from build123d import *

# Parameters (mm, degrees)
SKETCH1_W             = 12
SKETCH1_H             = 43.5
BOSS_EXTRUDE1_DEPTH   = 2
M3_TAPPED_HOLE1_D     = 2.5
M3_TAPPED_HOLE1_DEPTH = 7.5
M3_TAPPED_HOLE1_TIP   = 0.751075774
SKETCH6_W             = 25
SKETCH6_H             = 12
BOSS_EXTRUDE2_DEPTH   = 14
SKETCH7_W             = 25
SKETCH7_H             = 8
CUT_EXTRUDE4_DEPTH    = 32.273990791
SKETCH8_R             = 2.5
CUT_EXTRUDE5_DEPTH    = 15
SKETCH9_W             = 13
SKETCH9_H             = 4
SKETCH9_W_2           = 10
SKETCH9_H_2           = 6
CUT_EXTRUDE6_DEPTH    = 18
CHAMFER2_SIZE         = 2
FILLET1_R             = 2
FILLET2_R             = 2
SKETCH3_W             = 8
SKETCH3_H             = 8
CUT_EXTRUDE2_DEPTH    = 10
SKETCH10_R            = 0.25
CUT_EXTRUDE7_DEPTH    = 10
CUT_EXTRUDE8_DEPTH    = 10


with BuildPart() as part:
    # Sketch1 → Boss-Extrude1 (new body)
    with BuildSketch(Plane(origin=(0, 0, 0), x_dir=(1, 0, 0), z_dir=(0, 1, 0))):
        Rectangle(SKETCH1_W, SKETCH1_H)
    extrude(amount=BOSS_EXTRUDE1_DEPTH)

    # M3 Tapped Hole1
    with Locations(Plane(origin=(0, 2, 17.75), x_dir=(0, 0, 1), z_dir=(0, 1, 0))):
        with Locations((0, 0)):
            Hole(M3_TAPPED_HOLE1_D / 2, depth=M3_TAPPED_HOLE1_DEPTH)
            with Locations((0, 0, -(M3_TAPPED_HOLE1_DEPTH + M3_TAPPED_HOLE1_TIP / 2))):  # 118° drill point
                Cone(0, M3_TAPPED_HOLE1_D / 2, M3_TAPPED_HOLE1_TIP, mode=Mode.SUBTRACT)

    # Sketch6 → Boss-Extrude2 (add)
    with BuildSketch(Plane.XY.offset(21.75)):
        with Locations((-6.5, -4)):
            Rectangle(SKETCH6_W, SKETCH6_H)
    extrude(amount=-BOSS_EXTRUDE2_DEPTH)

    # Sketch7 → Cut-Extrude4 (cut, through all)
    with BuildSketch(Plane(origin=(0, 2, 0), x_dir=(1, 0, 0), z_dir=(0, 1, 0))):
        with Locations((-6.5, -17.75)):
            Rectangle(SKETCH7_W, SKETCH7_H)
    extrude(amount=-CUT_EXTRUDE4_DEPTH, mode=Mode.SUBTRACT)

    # Sketch8 → Cut-Extrude5 (cut)
    with BuildSketch(Plane.XY.offset(13.75)):
        with Locations((-14.5, -6)):
            Circle(SKETCH8_R)
    extrude(amount=-CUT_EXTRUDE5_DEPTH, mode=Mode.SUBTRACT)

    # Sketch9 → Cut-Extrude6 (cut)
    with BuildSketch(Plane.XY.offset(13.75)):
        with Locations((-12.5, 0)):
            Rectangle(SKETCH9_W, SKETCH9_H)
        with Locations((1, -7)):
            Rectangle(SKETCH9_W_2, SKETCH9_H_2)
    extrude(amount=-CUT_EXTRUDE6_DEPTH, mode=Mode.SUBTRACT)

    # Chamfer2
    chamfer2_edges = [part.edges().sort_by_distance(p)[0] for p in [
        (-19, -10, 10.75),
        (-19, -2, 10.75),
        (6, -4, 10.75),
        (-4, -10, 10.75),
    ]]
    chamfer(chamfer2_edges, length=CHAMFER2_SIZE)

    # Fillet1
    fillet1_edges = [part.edges().sort_by_distance(p)[0] for p in [
        (-4, -4, 10.75),
        (-6, -2, 10.75),
    ]]
    fillet(fillet1_edges, radius=FILLET1_R)

    # Fillet2
    fillet2_edges = [part.edges().sort_by_distance(p)[0] for p in [
        (-6, 1, -21.75),
        (6, 1, -21.75),
    ]]
    fillet(fillet2_edges, radius=FILLET2_R)

    # Sketch3 → Cut-Extrude2 (cut)
    with BuildSketch(Plane(origin=(0, 2, 0), x_dir=(1, 0, 0), z_dir=(0, 1, 0))):
        with Locations((0, 14.05)):
            Rectangle(SKETCH3_W, SKETCH3_H)
    extrude(amount=-CUT_EXTRUDE2_DEPTH, mode=Mode.SUBTRACT)

    # Sketch10 → Cut-Extrude7 (cut)
    with BuildSketch(Plane(origin=(0, 2, 0), x_dir=(1, 0, 0), z_dir=(0, 1, 0))):
        with Locations((-4, 10.05)):
            Circle(SKETCH10_R)
        with Locations((4, 10.05)):
            Circle(SKETCH10_R)
        with Locations((-4, 18.05)):
            Circle(SKETCH10_R)
        with Locations((4, 18.05)):
            Circle(SKETCH10_R)
    extrude(amount=-CUT_EXTRUDE7_DEPTH, mode=Mode.SUBTRACT)

    # Sketch11 → Cut-Extrude8 (cut)
    with BuildSketch(Plane.XY.offset(13.75)):
        with BuildLine():
            Line((-12, -5.4), (-12, -6.6))
            ThreePointArc((-12, -6.6), (-14.5, -9.1), (-17, -6.6))
            Line((-17, -6.6), (-17, -5.4))
            ThreePointArc((-17, -5.4), (-14.5, -2.9), (-12, -5.4))
        make_face()
    extrude(amount=-CUT_EXTRUDE8_DEPTH, mode=Mode.SUBTRACT)


solid = part.part
Source: CAD feature listing. Evaluate the final solid. Frame: model axes, mm. A direction names the side the tool comes from. Give positions to 0.01 mm unless a question says otherwise; leave off trailing zeros. Loops run counter-clockwise (first coordinate to the right, second up) from the corner with the lowest first, then second, coordinate; pieces in that order, holes last. Notation, with made-up numbers: (83, 43.25) -> (110, 43.25) arc R23 cw to (110, 63.25) -> close; hole circle Ø1 at (-27, 2.5). An arc over 180 degrees is marked (long way). Use a Markdown table: item, result. Add a question column.
1) Section query B-B, the plane y = 1. Return the cut outline in (x, z), then the cut area to 3 significant figures.
2) Section query C-C, the plane x = 2.5. Return the cut outline in (y, z), then the cut area to 3 significant figures.
3) Pull-direction query (Z, two-part tool) for faces 1 (the face through (0, 1, -21.75)), 2 (the face through (0, 2, -4)), 3 (the face through (-4, 1, -14)); classes: +Z half, -Z half, draft (parallel to the pull), parting line (faces both ways), or undercut.
4) Section query D-D, the plane y = -5. Return the cut outline in (x, z).
5) Section query A-A, the plane x = -14.5. Return the cut outline in (y, z).
6) First-contact query: pin 1 (1 mm diameter, centred on y = -7, z = 10.5, fed in from +X); pin 2 (3 mm diameter, centred on x = 0, z = 11.5, fed in from -Y); pin 3 (1 mm diameter, centred on y = 1, z = 3, fed in from -X). Flat tips, straight axial feed; report the tip coordinate or a pass-through.
7) Line query: line 1 along Y through (x, z) = (-2.25, 3); line 2 along X through (y, z) = (-6.5, 10.5); line 3 along Y through (x, z) = (-2, 12.5). Output: solid intervals per line, ascending. Write a range as [from, to].
8) Reachability of faces 4 (the face through (-12, -6, 11)), 5 (the face through (0, 0, -4)), 6 (the face through (-6, 1, -3)), 7 (the face through (0, 1, -18.05)), 8 (the face through (-4, -7, 11)) from +Z, -Z, +X, -X, +Y, -Y: full face, straight path, thin tool, end or side. Return the list, or none.
Numbers:
| question | item | result |
|---|---|---|
| 1 | outline | (-6, -19.75) arc R2 ccw to (-4, -21.75) -> (4, -21.75) arc R2 ccw to (6, -19.75) -> (6, 13.75) -> (-6, 13.75) -> close; hole (-4, -17.8) arc R0.25 ccw (long way) to (-3.75, -18.05) -> (3.75, -18.05) arc R0.25 ccw (long way) to (4, -17.8) -> (4, -10.3) arc R0.25 ccw (long way) to (3.75, -10.05) -> (-3.75, -10.05) arc R0.25 ccw (long way) to (-4, -10.3) -> close |
| 1 | area | 360 mm2 |
| 2 | outline | (-4, 7.75) -> (0, 7.75) -> (0, -10.05) -> (2, -10.05) -> (2, 13.75) -> (-4, 13.75) -> close; (0, -21.75) -> (2, -21.75) -> (2, -18.05) -> (0, -18.05) -> close |
| 2 | area | 79.0 mm2 |
| 3 | face 1 | -Z half |
| 3 | face 2 | draft |
| 3 | face 3 | undercut |
| 4 | outline | (-19, 7.75) -> (-16.97, 7.75) -> (-16.97, 13.75) -> (-19, 13.75) -> close; (-12.03, 7.75) -> (-3.73, 7.75) -> (-3.73, 13.75) -> (-12.03, 13.75) -> close |
| 5 | outline | (-10, 7.75) -> (-9.1, 7.75) -> (-9.1, 13.75) -> (-10, 13.75) -> close; (-2.9, 7.75) -> (-2, 7.75) -> (-2, 13.75) -> (-2.9, 13.75) -> close |
| 6 | pin 1 | stops at x = -4 |
| 6 | pin 2 | stops at y = -4 |
| 6 | pin 3 | stops at x = -6 |
| 7 | line 1 | y = [0, 2] |
| 7 | line 2 | x = [-19, -17], [-12, -4] |
| 7 | line 3 | y = [-4, 2] |
| 8 | face 4 | +Z, -Z |
| 8 | face 5 | -Z, +X, -X, -Y |
| 8 | face 6 | +Z, -Z, -X, +Y |
| 8 | face 7 | +Y, -Y |
| 8 | face 8 | +Z, -Z, +X, -Y |
